Design review of the part built by this model. Coordinates are the model's own, in mm. A direction names the side the tool comes from. Give positions to 0.01 mm unless a question says otherwise; leave off trailing zeros. Order: outer loops, then holes, each group sorted by start corner. A loop starts at its lowest first (then second) coordinate and runs counter-clockwise, first axis right, second up.
```python
from build123d import *
from OCP.BRepFilletAPI import BRepFilletAPI_MakeChamfer

# Parameters (mm, degrees)
SKETCH1_W                                            = 68
SKETCH1_H                                            = 87
BOSS_EXTRUDE1_DEPTH                                  = 12
SKETCH3_R                                            = 11
SKETCH3_W                                            = 32
SKETCH3_H                                            = 26
CUT_EXTRUDE2_DEPTH                                   = 57.5
CUT_EXTRUDE5_DEPTH                                   = 2
FILLET1_R                                            = 10
CHAMFER1_SIZE                                        = 2
CUT_EXTRUDE6_DEPTH                                   = 57.5
CHAMFER2_SIZE                                        = 12
CHAMFER2_SIZE2                                       = 4
FILLET3_R                                            = 0.5
HOLE_SIZE_BY_SOCKET_HEAD_CAP_SCREW_TYPE1_D           = 4.5
HOLE_SIZE_BY_SOCKET_HEAD_CAP_SCREW_TYPE1_CBORE_D     = 8
HOLE_SIZE_BY_SOCKET_HEAD_CAP_SCREW_TYPE1_CBORE_DEPTH = 4.6
SKETCH15_R                                           = 2
CUT_EXTRUDE4_DEPTH                                   = 25
CHAMFER3_SIZE                                        = 0.5


with BuildPart() as part:
    # Sketch1 → Boss-Extrude1 (new body)
    with BuildSketch(Plane.XY):
        Rectangle(SKETCH1_W, SKETCH1_H)
    extrude(amount=BOSS_EXTRUDE1_DEPTH)

    # Sketch3 → Cut-Extrude2 (cut, through all)
    with BuildSketch(Plane.XY.offset(12)):
        Circle(SKETCH3_R)
        with Locations((-18, 30.5)):
            Rectangle(SKETCH3_W, SKETCH3_H)
        with Locations((18, -30.5)):
            Rectangle(SKETCH3_W, SKETCH3_H)
    extrude(amount=-CUT_EXTRUDE2_DEPTH, mode=Mode.SUBTRACT)

    # Sketch16 → Cut-Extrude5 (cut)
    with BuildSketch(Plane.XY.offset(12)):
        with BuildLine():
            Line((0, -43.5), (-32, -43.5))
            Line((-32, -43.5), (-32, -26))
            ThreePointArc((-32, -26), (-33.060660172, -23.439339828), (-30.5, -24.5))
            Line((-30.5, -24.5), (-1.5, -24.5))
            ThreePointArc((-1.5, -24.5), (1.060660172, -23.439339828), (0, -26))
            Line((0, -26), (0, -43.5))
        make_face()
        with BuildLine():
            Line((32, 43.5), (0, 43.5))
            Line((0, 43.5), (0, 26))
            ThreePointArc((0, 26), (-1.060660172, 23.439339828), (1.5, 24.5))
            Line((1.5, 24.5), (30.5, 24.5))
            ThreePointArc((30.5, 24.5), (33.060660172, 23.439339828), (32, 26))
            Line((32, 26), (32, 43.5))
        make_face()
    extrude(amount=-CUT_EXTRUDE5_DEPTH, mode=Mode.SUBTRACT)

    # Fillet1
    fillet1_edges = [part.edges().sort_by_distance(p)[0] for p in [
        (-2, 17.5, 6),
        (2, -17.5, 6),
    ]]
    fillet(fillet1_edges, radius=FILLET1_R)

    # Chamfer1
    chamfer1_edges = [part.edges().sort_by_distance(p)[0] for p in [
        (-34, -43.5, 6),
        (2, -43.5, 6),
        (34, 43.5, 6),
        (-2, 43.5, 6),
    ]]
    chamfer(chamfer1_edges, length=CHAMFER1_SIZE)

    # Sketch17 → Cut-Extrude6 (cut, through all)
    with BuildSketch(Plane(origin=(0, 0, 0), x_dir=(-1, 0, 0), z_dir=(0, 0, -1))):
        with BuildLine():
            Line((-20.75, 36.5), (-20.75, 31.5))
            ThreePointArc((-20.75, 31.5), (-23.5, 28.75), (-26.25, 31.5))
            Line((-26.25, 31.5), (-26.25, 36.5))
            ThreePointArc((-26.25, 36.5), (-23.5, 39.25), (-20.75, 36.5))
        make_face()
        with BuildLine():
            Line((-5.75, 36.5), (-5.75, 31.5))
            ThreePointArc((-5.75, 31.5), (-8.5, 28.75), (-11.25, 31.5))
            Line((-11.25, 31.5), (-11.25, 36.5))
            ThreePointArc((-11.25, 36.5), (-8.5, 39.25), (-5.75, 36.5))
        make_face()
        with BuildLine():
            Line((26.25, -31.5), (26.25, -36.5))
            ThreePointArc((26.25, -36.5), (23.5, -39.25), (20.75, -36.5))
            Line((20.75, -36.5), (20.75, -31.5))
            ThreePointArc((20.75, -31.5), (23.5, -28.75), (26.25, -31.5))
        make_face()
        with BuildLine():
            Line((11.25, -31.5), (11.25, -36.5))
            ThreePointArc((11.25, -36.5), (8.5, -39.25), (5.75, -36.5))
            Line((5.75, -36.5), (5.75, -31.5))
            ThreePointArc((5.75, -31.5), (8.5, -28.75), (11.25, -31.5))
        make_face()
    extrude(amount=-CUT_EXTRUDE6_DEPTH, mode=Mode.SUBTRACT)

    # Chamfer2: one chamfer whose edges measure the first distance from different faces: ONE call of the kernel's chamfer builder (chamfer() names one face for all edges)
    chamfer2_edges_1 = [part.edges().sort_by_distance(p)[0] for p in [
        (-34, 17.5, 6),
    ]]
    chamfer2_side_1 = [part.faces().sort_by_distance(p)[0] for p in [
        (-34, -12, 6),
    ]]
    chamfer2_edges_2 = [part.edges().sort_by_distance(p)[0] for p in [
        (34, -17.5, 6),
    ]]
    chamfer2_side_2 = [part.faces().sort_by_distance(p)[0] for p in [
        (34, 12, 6),
    ]]
    chamfer2 = BRepFilletAPI_MakeChamfer(part.part.solid().wrapped)
    for e in chamfer2_edges_1:
        chamfer2.Add(CHAMFER2_SIZE, CHAMFER2_SIZE2, e.wrapped, chamfer2_side_1[0].wrapped)  # the first distance lies on this face
    for e in chamfer2_edges_2:
        chamfer2.Add(CHAMFER2_SIZE, CHAMFER2_SIZE2, e.wrapped, chamfer2_side_2[0].wrapped)  # the first distance lies on this face
    add(Compound.cast(chamfer2.Shape()), mode=Mode.REPLACE)

    # Fillet3
    fillet3_edges = [part.edges().sort_by_distance(p)[0] for p in [
        (30, -17.5, 6),
        (34, -5.5, 6),
        (-30, 17.5, 6),
        (-34, 5.5, 6),
    ]]
    fillet(fillet3_edges, radius=FILLET3_R)

    # Hole size by socket head cap screw type1 (through all)
    with Locations(Plane.XY.offset(12)):
        with Locations((17.5, 12.5), (-17.5, -12.5)):
            CounterBoreHole(HOLE_SIZE_BY_SOCKET_HEAD_CAP_SCREW_TYPE1_D / 2, HOLE_SIZE_BY_SOCKET_HEAD_CAP_SCREW_TYPE1_CBORE_D / 2, HOLE_SIZE_BY_SOCKET_HEAD_CAP_SCREW_TYPE1_CBORE_DEPTH)

    # Sketch15 → Cut-Extrude4 (cut)
    with BuildSketch(Plane.XY.offset(12)):
        with Locations((17.5, -12.5)):
            Circle(SKETCH15_R)
        with Locations((-17.5, 12.5)):
            Circle(SKETCH15_R)
    extrude(amount=-CUT_EXTRUDE4_DEPTH, mode=Mode.SUBTRACT)

    # Chamfer3
    chamfer3_edges = [part.edges().sort_by_distance(p)[0] for p in [
        (-11, 0, 0),
        (-11, 0, 12),
    ]]
    chamfer(chamfer3_edges, length=CHAMFER3_SIZE)


solid = part.part
```
1. For line 1 along X through (y, z) = (-33.5, 6.5); line 2 along Y through (x, z) = (17.5, 7.5); line 3 along Y through (x, z) = (-17.5, 9.15), list the stretches that pass through material, from the lowest coordinate up.
Recorded:
line 1: x = -34 to -26.25, -20.75 to -11.25, -5.75 to 2
line 2: y = -17.5 to -14.5, -10.5 to 8.5, 16.5 to 43.5
line 3: y = -43.5 to -16.5, -8.5 to 10.5, 14.5 to 17.5
2. Draft analysis for pull direction X (two halves, no side actions). For faces 1 (the face through (21, -17.5, 6)), 2 (the face through (-2, 34, 6)), 3 (the face through (5.75, 34, 5)), state which applies: pulls with the +X half, pulls with the -X half, needs draft (parallel to the pull), parting line crosses it, or undercut.
Recorded:
face 1: needs draft
face 2: pulls with the -X half
face 3: undercut
3. Take a section at B-B (y = -13.5). State the section outline as (x, z) points.
Recorded:
outline: (-34, 0) - (-19.52, 0) - (-19.52, 7.4) - (-21.37, 7.4) - (-21.37, 12) - (-34, 12) - close; (-15.48, 0) - (15.77, 0) - (15.77, 12) - (-13.63, 12) - (-13.63, 7.4) - (-15.48, 7.4) - close; (19.23, 0) - (31.33, 0) - (31.33, 12) - (19.23, 12) - close
4. For pin 1 (2 mm diameter, centred on x = -14.5, z = 6, fed in from +Y); pin 2 (3.5 mm diameter, centred on x = 0, y = -24.5, fed in from +Z); pin 3 (4 mm diameter, centred on y = -33, z = 6, fed in from +X); pin 4 (4 mm diameter, centred on y = 34.5, z = 6.5, fed in from -X), all flat-tipped, find the tip position at first contact; note any pin that passes through.
Recorded:
pin 1: stops at y = 17.5
pin 2: stops at z = 12
pin 3: stops at x = 2
pin 4: stops at x = -2
5. Take a section at A-A (x = -27.5). State the section outline as (y, z) points, then the cut area to 3 significant figures.
Recorded:
outline: (-43.5, 0) - (17.5, 0) - (17.5, 12) - (-24.5, 12) - (-24.5, 10) - (-43.5, 10) - close
area: 694 mm2
6. Machinability: for faces 4 (the face through (2, -35, 6)), 5 (the face through (7, 10, 12)), 6 (the face through (-11.25, -34, 5)), 7 (the face through (-1.095, 23.475, 11.014)), which of the approach directions +Z, -Z, +X, -X, +Y, -Y give a long, thin tool a straight path to every point of the face, cutting with its end or side? Answer none if there is none.
Recorded:
face 4: +Z, -Z, +X, -Y
face 5: +Z, +X, -X, +Y, -Y
face 6: +Z, -Z
face 7: +Z
7. Take a section at C-C (z = 5.5). State how many separate pieces and enclosed holes the cut face has, then the cut area to 3 significant figures.
Recorded:
separate pieces: 1
enclosed holes: 9
area: 3,600 mm2
